Verification items for the finished model (mm, model axes). A direction names the side the tool comes from. Give positions to 0.01 mm unless a question says otherwise; leave off trailing zeros. Loops run counter-clockwise (first coordinate to the right, second up) from the corner with the lowest first, then second, coordinate; pieces in that order, holes last. Notation, with made-up numbers: M 38.5,6 L 61.5,6 A26 cw 61.5,32 Z; hole C -11.75,22.5 d6. An arc over 180 degrees is marked long. Put each result on its own line as item: value. Start each with the question number.
from build123d import *


with BuildPart() as part:
    # 草图1 → 旋转1 (revolve)
    with BuildSketch(Plane.XY, mode=Mode.PRIVATE) as revolve_1_sk:
        Polygon((1.25, 0), (4.5, 0), (3, 2), (3, 3.5), (3.5, 4.37), (3.5, 12), (1.25, 12), align=None)
    revolve(revolve_1_sk.sketch.rotate(Axis((0, 0, 0), (0, 1, 0)), 270), axis=Axis((0, 0, 0), (0, 1, 0)))


solid = part.part
Q1. Set-up check for faces 4 (the face through (-3.417, 8.238, -0.759)), 5 (the face through (-2, 12, 0)): record each of +Z, -Z, +X, -X, +Y, -Y from which the full face is reachable in a straight line by a thin tool's end or side.
Q2. Release check for a two-part mould opening along Y. For faces 1 (the face through (-1.22, 5.92, -0.27)), 2 (the face through (-1, 0, -1)), 3 (the face through (0.9, 2.76, 2.86)) record: pulls with the +Y half, pulls with the -Y half, needs draft (parallel to the pull), parting line crosses it, or undercut.
Q3. Cross-section at B-B, the plane z = 0. Record the boundary of the cut face in (x, y).
Q4. Cross-section at D-D, the plane y = 2.5. Record the boundary of the cut face in (x, z), then the cut area to 3 significant figures.
Q5. Go/stop test with flat-tipped pins: pin 1 (1.5 mm diameter, centred on x = 0.5, y = 9.5, fed in from -Z); pin 2 (4 mm diameter, centred on x = -0.5, y = 2.5, fed in from +Z); pin 3 (2 mm diameter, centred on x = -0.5, z = 0, fed in from +Y); pin 4 (4 mm diameter, centred on y = 7.5, z = 2, fed in from +X). Record where each tip stops, or that it passes through.
Q6. Cross-section at A-A, the plane x = 0. Record the boundary of the cut face in (y, z), then the cut area to 3 significant figures.
Q7. Cross-section at C-C, the plane y = 6. Record the boundary of the cut face in (x, z).
Q8. Scan lines: L1, parallel to X at y = 6.75, z = 0; L2, parallel to X at y = 2.75, z = 0; L3, parallel to Y at x = 0.75, z = -3. Record each from-to range of solid material in increasing order.
Ans:
1. face 4: +Y
1. face 5: +Z, -Z, +X, -X, +Y
2. face 1: needs draft
2. face 2: pulls with the -Y half
2. face 3: undercut
3. outline: M -4.5,0 L -1.25,0 L -1.25,12 L -3.5,12 L -3.5,4.37 L -3,3.5 L -3,2 Z; M 1.25,0 L 4.5,0 L 3,2 L 3,3.5 L 3.5,4.37 L 3.5,12 L 1.25,12 Z
4. outline: C 0,0 d6; hole C 0,0 d2.5
4. area: 23.4 mm^2
5. pin 1: stops at z = -3.5
5. pin 2: stops at z = 4.11
5. pin 3: stops at y = 12
5. pin 4: stops at x = 3.5
6. outline: M 0,-4.5 L 2,-3 L 3.5,-3 L 4.37,-3.5 L 12,-3.5 L 12,-1.25 L 0,-1.25 Z; M 0,1.25 L 12,1.25 L 12,3.5 L 4.37,3.5 L 3.5,3 L 2,3 L 0,4.5 Z
6. area: 53.1 mm^2
7. outline: C 0,0 d7; hole C 0,0 d2.5
8. L1: x = -3.5 to -1.25, 1.25 to 3.5
8. L2: x = -3 to -1.25, 1.25 to 3
8. L3: y = 0 to 1.88, 3.66 to 12
